```python
from build123d import *

# Parameters (mm, degrees)
EXTRUDE_1_DEPTH      = 40
EXTRUDE_1_DEPTH_BACK = 40
SKETCH_1_R           = 25
SKETCH_1_R_2         = 15
EXTRUDE_2_DEPTH      = 10
EXTRUDE_2_DEPTH_BACK = 10
SKETCH_3_R           = 12.5
SKETCH_3_R_2         = 10
EXTRUDE_3_DEPTH      = 30
SKETCH_4_R           = 25
SKETCH_4_R_2         = 75
BOSS_EXTRUDE4_DEPTH  = 20
SKETCH_5_R           = 9
BOSS_EXTRUDE5_DEPTH  = 15


with BuildPart() as part:
    # 草图1 → 凸台-拉伸1 (new, two sides: drawn at the far end of the back side and taken through both)
    with BuildSketch(Plane.XY.offset(-EXTRUDE_1_DEPTH_BACK)):
        Circle(SKETCH_1_R)
        Circle(SKETCH_1_R_2, mode=Mode.SUBTRACT)
    extrude(amount=EXTRUDE_1_DEPTH + EXTRUDE_1_DEPTH_BACK)

    # 草图2 → 凸台-拉伸2 (add, two sides: drawn at the far end of the back side and taken through both)
    with BuildSketch(Plane.XY.offset(-EXTRUDE_2_DEPTH_BACK)):
        with BuildLine():
            Line((-11.804411719, -22.037601139), (86.449952125, -59.348644826))
            ThreePointArc((86.449952125, -59.348644826), (89.473468939, -59.986128631), (92.547259147, -59.670132928))
            Line((92.547259147, -59.670132928), (273.184073933, -12.08766616))
            ThreePointArc((273.184073933, -12.08766616), (282.19931165, 2.725214721), (267.737534205, 12.293544994))
            Line((267.737534205, 12.293544994), (174.388702716, -4.886083694))
            Line((174.388702716, -4.886083694), (86.450111626, -12.08766616))
            Line((86.450111626, -12.08766616), (7.341932544, 23.897615499))
            ThreePointArc((7.341932544, 23.897615499), (20.013015277, -8.341662634), (-11.804411719, -22.037601139))
        make_face()
    extrude(amount=EXTRUDE_2_DEPTH + EXTRUDE_2_DEPTH_BACK)

    # 草图3 → 凸台-拉伸3 (add)
    with BuildSketch(Plane.XY.offset(10)):
        with Locations((270, 0)):
            Circle(SKETCH_3_R)
        with Locations((90, -50)):
            Circle(SKETCH_3_R_2)
    extrude(amount=EXTRUDE_3_DEPTH)

    # 草图4 → Boss-Extrude4 (add)
    with BuildSketch(Plane.XY.offset(15)):
        with Locations((90, -50)):
            Circle(SKETCH_4_R)
        with Locations((270, 0)):
            Circle(SKETCH_4_R_2)
    extrude(amount=BOSS_EXTRUDE4_DEPTH)

    # 草图5 → Boss-Extrude5 (add)
    with BuildSketch(Plane.XY.offset(10)):
        with BuildLine():
            Line((120.752986945, -33.386484264), (109.111101455, 19.729618285))
            ThreePointArc((109.111101455, 19.729618285), (121.314568975, 38.784155291), (140.36910598, 26.58068777))
            Line((140.36910598, 26.58068777), (152.010991471, -26.535414779))
            Line((152.010991471, -26.535414779), (120.752986945, -33.386484264))
        make_face()
        with Locations((124.740103717, 23.155153028)):
            Circle(SKETCH_5_R, mode=Mode.SUBTRACT)
    extrude(amount=BOSS_EXTRUDE5_DEPTH)

    # Mirror2: part across plane


with BuildPart() as part_1:
    add(part.part)
    add(part.part.mirror(Plane.XY))


solid = part_1.part
```
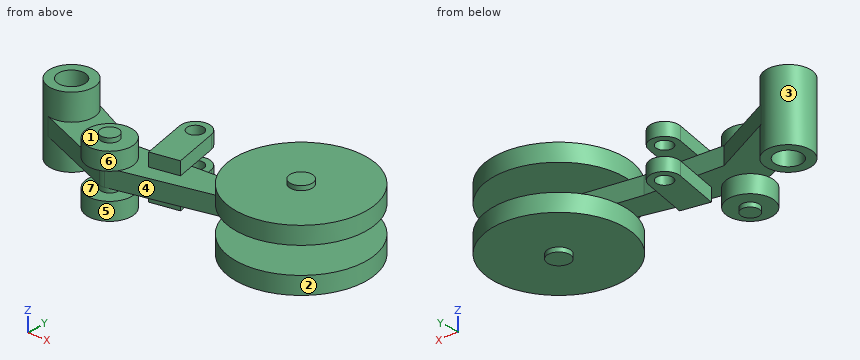
CAD build for the part. Positions are in the model's coordinates, mm. Face numbers are marked on the shaded views. A direction names the side the tool comes from. Give positions to 0.01 mm unless a question says otherwise; leave off trailing zeros. Order: outer loops, then holes, each group sorted by start corner. A loop starts at its lowest first (then second) coordinate and runs counter-clockwise, first axis right, second up.
(1) Tool access for the marked faces 5, 6 and 7: list every direction of +Z, -Z, +X, -X, +Y, -Y with a clear straight run to the whole face (end or side of a thin tool).
(2) Saw through at C-C, the plane z = 3.5. Give the cut face in (x, y).
(3) Mould opens along X. For the marked faces 1, 2, 3 and 4 say: released by +X, released by -X, zero draft, split by the parting line, or undercut.
(4) Saw through at D-D, the plane x = 0. Give the cut face in (y, z).
(5) Saw through at A-A, the plane y = 51.5. Give the cut face in (x, z), then the cut area to 3 significant figures.
(6) Drill centre lines: L1, parallel to Z at x = 262.5, y = -13.5; L2, parallel to Z at x = 255.5, y = 27.5; L3, parallel to X at y = -6, z = -20. Where is each one in solid material? Low to high.
(7) Flat gauge pins, fed straight in: pin 1 (1 mm diameter, centred on x = 146.5, y = -23, fed in from +Z); pin 2 (10 mm diameter, centred on y = -59, z = 17, fed in from +X); pin 3 (12 mm diameter, centred on y = -7.5, z = 24.5, fed in from -X). Where does each tip first touch, or does it go through?
(8) Saw through at B-B, the plane x = 126. Give the cut face in (y, z), then the cut area to 3 significant figures.
Results found:
1. face 5: -Z
1. face 6: +Z
1. face 7: none
2. outline: (-5.8, -24.32) - (86.45, -59.35) arc R10 ccw to (92.55, -59.67) - (273.18, -12.09) arc R12.5 ccw to (267.74, 12.29) - (174.39, -4.89) - (86.45, -12.09) - (13.19, 21.24) arc R25 ccw (long way) to start; hole circle Ø30 at (0, 0)
3. face 1: zero draft
3. face 2: undercut
3. face 3: undercut
3. face 4: released by +X
4. outline: (-26.52, -10) - (-25, -10) - (-25, -40) - (-15, -40) - (-15, 40) - (-25, 40) - (-25, 10) - (-26.52, 10) - close; (15, -40) - (25, -40) - (25, 40) - (15, 40) - close
5. outline: (215.48, -35) - (324.52, -35) - (324.52, -15) - (215.48, -15) - close; (215.48, 15) - (324.52, 15) - (324.52, 35) - (215.48, 35) - close
5. area: 4,360 mm2
6. L1: z = -35 to -15, -10 to 10, 15 to 35
6. L2: z = -35 to -15, 15 to 35
6. L3: x = -24.27 to -13.75, 13.75 to 24.27, 114.75 to 147.51, 195.24 to 344.76
7. pin 1: stops at z = 25
7. pin 2: stops at x = 322.05
7. pin 3: stops at x = -24.95
8. outline: (-50.86, -10) - (-32.24, -10) - (-32.24, -25) - (14.24, -25) - (14.24, -10) - (-8.85, -10) - (-8.85, 10) - (14.24, 10) - (14.24, 25) - (-32.24, 25) - (-32.24, 10) - (-50.86, 10) - close; (32.07, -25) - (39.11, -25) - (39.11, -10) - (32.07, -10) - close; (32.07, 10) - (39.11, 10) - (39.11, 25) - (32.07, 25) - close
8. area: 2,450 mm2
